For this review, use the dimensioned drawing (mm, ordinates from the lowest corner) and the shaded views. A direction names the side the tool comes from. Coordinates: 2 decimals unless noted, no trailing zeros. Order: outer loops, then holes, each group sorted by start corner. A loop starts at its lowest first (then second) coordinate and runs counter-clockwise, first axis right, second up. Notation, with made-up numbers: M 85.5,26 L 103.5,26 A19 ccw 103.5,58 Z; hole C 69.25,49 d4. An arc over 180 degrees is marked long. Use CSV: the item, a comma, the result in double quotes.
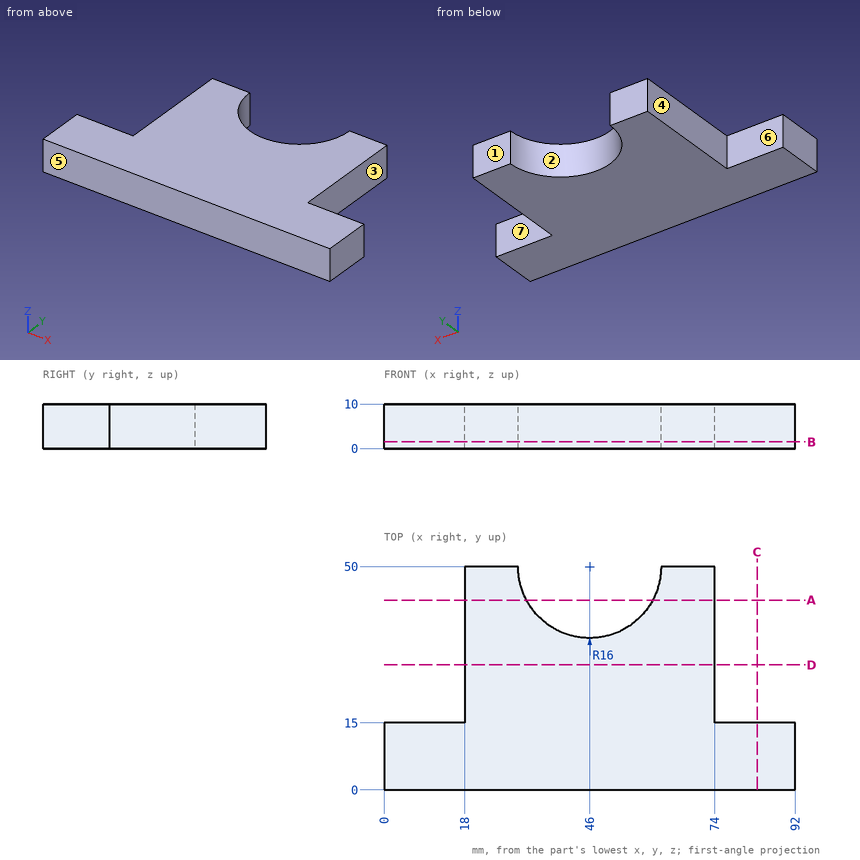
Item 1: Add section A-A on y = 42.5. State the section outline as (x, z) points, and give its area (3 significant figures).
Solutions:
outline,"M 18,0 L 31.87,0 L 31.87,10 L 18,10 Z; M 60.13,0 L 74,0 L 74,10 L 60.13,10 Z"
area,"277 mm^2"
Item 2: Clearance check with flat-ended pins moving along their axes: pin 1 Ø4 at (y, z) = (10, 5) entering from -X; pin 2 Ø2 at (y, z) = (25, 5.5) entering from -X; pin 3 Ø5 at (y, z) = (37.5, 6) entering from +X; pin 4 Ø1.5 at (x, z) = (50.5, 8) entering from +Y. State where each tip first meets the part, or that it passes through.
Solutions:
pin 1,"x = 0"
pin 2,"x = 18"
pin 3,"x = 74"
pin 4,"y = 34.89"
Item 3: To check wall thickness, follow line 1 along X through (y, z) = (38, 3.5); line 2 along X through (y, z) = (37, 3); line 3 along X through (y, z) = (30, 6.75). State the ranges of each line that lie inside material, in increasing order. Write a range as [from, to].
Solutions:
line 1,"[18, 35.42], [56.58, 74]"
line 2,"[18, 36.67], [55.33, 74]"
line 3,"[18, 74]"
Item 4: Add section C-C on x = 83.5. State the section outline as (y, z) points.
Solutions:
outline,"M 0,0 L 15,0 L 15,10 L 0,10 Z"
Item 5: For the marked faces 5, 6 and 7, list the 3-axis set-ups (+Z, -Z, +X, -X, +Y, -Y) from which the entire face can be reached by the end or side of a thin tool; tool diameter is ignored.
Solutions:
face 5,"+Z, -Z, +X, -X, -Y"
face 6,"+Z, -Z, -X, +Y"
face 7,"+Z, -Z, +X, +Y"
Item 6: Draft analysis for pull direction X (two halves, no side actions). For the marked faces 1, 2, 3 and 4, state which applies: released by +X, released by -X, zero draft, split by the parting line, or undercut.
Solutions:
face 1,"zero draft"
face 2,"undercut"
face 3,"released by +X"
face 4,"released by -X"
Item 7: Add section D-D on y = 28. State the section outline as (x, z) points, and give its area (3 significant figures).
Solutions:
outline,"M 18,0 L 74,0 L 74,10 L 18,10 Z"
area,"560 mm^2"
Item 8: Add section B-B on z = 1.5. State the section outline as (x, y) points.
Solutions:
outline,"M 0,0 L 92,0 L 92,15 L 74,15 L 74,50 L 62,50 A16 cw 30,50 L 18,50 L 18,15 L 0,15 Z"
